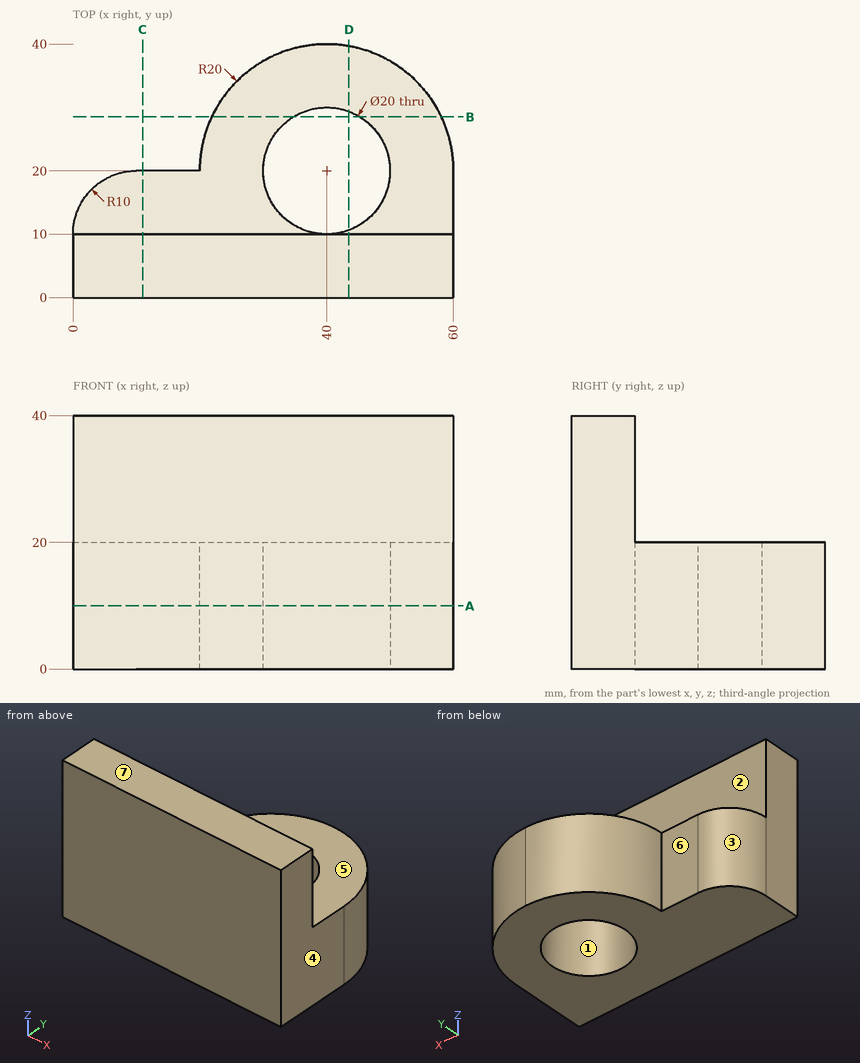
For this review, use the dimensioned drawing (mm, ordinates from the lowest corner) and the shaded views. A direction names the side the tool comes from. Give positions to 0.01 mm unless a question says otherwise; leave off trailing zeros. Order: outer loops, then holes, each group sorted by start corner. A loop starts at its lowest first (then second) coordinate and runs counter-clockwise, first axis right, second up. Notation, with made-up numbers: (68.5, 3) -> (124.5, 3) arc R22 cw to (124.5, 16) -> close; hole circle Ø2 at (87, -23.5). An arc over 180 degrees is marked (long way). Write item = value, one per line. Start each with the question number.
(1) Take a section at A-A (z = 10). Write out the cut boundary in (x, y), plus the area to 3 significant figures.
(2) For L1, parallel to Y at x = 18.5, z = 4; L2, parallel to X at y = 11, z = 5.5; L3, parallel to Y at x = 24.5, z = 27, list the stretches that pass through material, from the lowest coordinate up. Write a range as from..to.
(3) For pin 1 Ø3 at (x, z) = (14, 11.5) entering from +Y; pin 2 Ø4 at (x, z) = (36, 33) entering from +Y; pin 3 Ø18 at (x, y) = (40, 20) entering from -Z; pin 4 Ø15 at (x, y) = (40.5, 31) entering from +Z, all flat-tipped, find the tip position at first contact; note any pin that passes through.
(4) Take a section at C-C (x = 11). Write out the cut boundary in (y, z), plus the area to 3 significant figures.
(5) Tool access review of the marked faces 5, 6 and 7: name each direction out of +Z, -Z, +X, -X, +Y, -Y from which nothing blocks a thin tool from reaching the whole face with its end or side.
(6) Draft analysis for pull direction X (two halves, no side actions). For the marked faces 1, 2, 3 and 4, state which applies: +X half, -X half, draft (parallel to the pull), parting line (faces both ways), or undercut.
(7) Take a section at D-D (x = 43.5). Write out the cut boundary in (y, z).
(8) Take a section at B-B (y = 28.5). Write out the cut boundary in (x, z), plus the area to 3 significant figures.
Returned:
q1.outline = (0, 0) -> (60, 0) -> (60, 20) arc R20 ccw to (20, 20) -> (10, 20) arc R10 ccw to (0, 10) -> close; hole circle Ø20 at (40, 20)
q1.area = 1,490 mm²
q2.L1 = 0..20
q2.L2 = 0.05..35.64, 44.36..60
q2.L3 = 0..10
q3.pin_1 = 20
q3.pin_2 = 10
q3.pin_3 = through
q3.pin_4 = 20
q4.outline = (0, 0) -> (20, 0) -> (20, 20) -> (10, 20) -> (10, 40) -> (0, 40) -> close
q4.area = 600 mm²
q5.face_5 = +Z, +X, -X, +Y
q5.face_6 = +Z, -Z, -X, +Y
q5.face_7 = +Z, +X, -X, +Y, -Y
q6.face_1 = undercut
q6.face_2 = draft
q6.face_3 = -X half
q6.face_4 = +X half
q7.outline = (0, 0) -> (10.63, 0) -> (10.63, 20) -> (10, 20) -> (10, 40) -> (0, 40) -> close; (29.37, 0) -> (39.69, 0) -> (39.69, 20) -> (29.37, 20) -> close
q8.outline = (21.9, 0) -> (34.73, 0) -> (34.73, 20) -> (21.9, 20) -> close; (45.27, 0) -> (58.1, 0) -> (58.1, 20) -> (45.27, 20) -> close
q8.area = 513 mm²
